The model under review builds one solid part; all positions refer to its coordinate system, in mm. A direction names the side the tool comes from. Coordinates: 2 decimals unless noted, no trailing zeros. Write each loop counter-clockwise with the first axis right and the second up, starting at its lowest first coordinate (ties: lowest second). Pieces come first, ordered by that corner, then holes. Notation, with made-up numbers: (73, 62.25) - (94, 62.25) arc R10 ccw to (94, 67.25) - close; hole circle Ø1 at (-38, 74.25). An arc over 180 degrees is marked (long way). Put each result on its own line as item: value. Start each with the question number.
Item 1: Consider section A-A on x = 606.5. Give the boundary of the cut face in (y, z).
Item 2: To check wall thickness, follow L1, parallel to X at y = 10.5, z = 1.75; L2, parallel to X at y = 29.4, z = 11; L3, parallel to Z at x = 260, y = 29.65. State the ranges of each line that lie inside material, in increasing order. Write a range as [from, to].
Item 3: Mouldability with a two-part tool opening along Z and no side actions: class faces 1 (the face through (414, 27, 0)), 2 (the face through (407, 30, 11)), 3 (the face through (1.5, 14, 11)) as pulls with the +Z half, pulls with the -Z half, needs draft (parallel to the pull), parting line crosses it, or undercut.
Item 4: For pin 1 (1.6 mm diameter, centred on x = 0.5, z = 9.5, fed in from +Y); pin 2 (1.5 mm diameter, centred on x = 354, y = 20.5, fed in from -Z); pin 3 (0.8 mm diameter, centred on x = 0.5, z = 9.5, fed in from +Y); pin 4 (0.6 mm diameter, centred on x = 476, z = 21, fed in from -Y), all flat-tipped, find the tip position at first contact; note any pin that passes through.
Item 5: Machinability: for faces 4 (the face through (0, 13, 11)), 5 (the face through (823.5, 14, 11)), which of the approach directions +Z, -Z, +X, -X, +Y, -Y give a long, thin tool a straight path to every point of the face, cutting with its end or side? Answer none if there is none.
```python
from build123d import *

# Parameters (mm, degrees)
EXTRUDE_1_DEPTH       = 22
SKETCH_2_W            = 822
SKETCH_2_H            = 6
EXTRUDE_2_DEPTH       = 2
SKETCH_3_W            = 822
SKETCH_3_H            = 6
EXTRUDE_3_DEPTH       = 2
CUT_EXTRUDE_1_DEPTH   = 826.838361909
CHAMFER_1_SIZE        = 2
FILLET_1_R            = 3
HOLE_WIZARD_7_0_7_1_D = 7


with BuildPart() as part:
    # 草图1 → 凸台-拉伸1 (new body)
    with BuildSketch(Plane.XY):
        Polygon((0, 0), (0, 30), (825, 30), (825, 0), (823.5, 0), (823.5, 28.5), (1.5, 28.5), (1.5, 0), align=None)
    extrude(amount=EXTRUDE_1_DEPTH)

    # 草图2 → 凸台-拉伸2 (add)
    with BuildSketch(Plane.XY.offset(22)):
        with Locations((412.5, 25.5)):
            Rectangle(SKETCH_2_W, SKETCH_2_H)
    extrude(amount=-EXTRUDE_2_DEPTH)

    # 草图3 → 凸台-拉伸3 (add)
    with BuildSketch(Plane(origin=(0, 0, 0), x_dir=(-1, 0, 0), z_dir=(0, 0, -1))):
        with Locations((-412.5, 25.5)):
            Rectangle(SKETCH_3_W, SKETCH_3_H)
    extrude(amount=-EXTRUDE_3_DEPTH)

    # 草图5 → 切除-拉伸1 (cut, through all)
    with BuildSketch(Plane.ZY):
        with BuildLine():
            Line((8, 20), (14, 20))
            ThreePointArc((14, 20), (16.5, 17.5), (14, 15))
            Line((14, 15), (8, 15))
            ThreePointArc((8, 15), (5.5, 17.5), (8, 20))
        make_face()
        with BuildLine():
            Line((8, 8), (14, 8))
            ThreePointArc((14, 8), (16.5, 5.5), (14, 3))
            Line((14, 3), (8, 3))
            ThreePointArc((8, 3), (5.5, 5.5), (8, 8))
        make_face()
    extrude(amount=-CUT_EXTRUDE_1_DEPTH, mode=Mode.SUBTRACT)

    # 倒角1
    chamfer_1_edges = [part.edges().sort_by_distance(p)[0] for p in [
        (0.75, 0, 0),
        (824.25, 0, 22),
        (0.75, 0, 22),
        (824.25, 0, 0),
    ]]
    chamfer(chamfer_1_edges, length=CHAMFER_1_SIZE)

    # 圆角1
    fillet_1_edges = [part.edges().sort_by_distance(p)[0] for p in [
        (0, 30, 11),
        (825, 30, 11),
    ]]
    fillet(fillet_1_edges, radius=FILLET_1_R)

    # Ø7.0 (7) 直径孔1 (through all)
    with Locations(Plane(origin=(0, 28.5, 0), x_dir=(-1, 0, 0), z_dir=(0, -1, 0))):
        with Locations((-100, -11), (-260, -11), (-420, -11), (-545, -11), (-725, -11)):
            Hole(HOLE_WIZARD_7_0_7_1_D / 2)


solid = part.part
```
Report:
1. outline: (22.5, 0) - (30, 0) - (30, 22) - (22.5, 22) - (22.5, 20) - (28.5, 20) - (28.5, 2) - (22.5, 2) - close
2. L1: [0, 1.5], [823.5, 825]
2. L2: [1.2, 96.5], [103.5, 256.5], [263.5, 416.5], [423.5, 541.5], [548.5, 721.5], [728.5, 823.8]
2. L3: [0, 7.5], [14.5, 22]
3. face 1: pulls with the -Z half
3. face 2: needs draft
3. face 3: undercut
4. pin 1: y = 29.47
4. pin 2: through
4. pin 3: y = 29.14
4. pin 4: y = 22.5
5. face 4: +Z, -Z, -X, +Y, -Y
5. face 5: -Y
